Could you check a few things on this model? Use its own coordinates, in mm. Face numbers are marked on the shaded views. A direction names the side the tool comes from. Round coordinates to 2 decimals unless told otherwise and drop trailing zeros. Write each loop counter-clockwise with the first axis right and the second up, starting at its lowest first coordinate (ties: lowest second). Pieces come first, ordered by that corner, then holes. Notation, with made-up numbers: M 33,-26 L 84,-26 A19 cw 84,5 Z; hole C 25,-35 d11. An arc over 180 degrees is marked long. One line per item, written item: value. Start each with the question number.
(1) If I drill on L1, parallel to Y at x = 0, z = -8; L2, parallel to Z at x = 16.5, y = -23.5; L3, parallel to X at y = -17, z = -6, over which ranges is the centre line in solid material (lowest first)?
(2) Which directions (+Z, -Z, +X, -X, +Y, -Y) give clear straight access to the entire face, cutting with the end or side of a thin tool? Please do the marked faces 5, 6, 7, 8 and 9.
(3) I'm going to push flat-ended pins straight in: pin 1 Ø13 at (x, y) = (30.31, 17.5) entering from +Z; pin 2 Ø1.5 at (x, z) = (-36.5, 2.5) entering from +Y; pin 3 Ø1 at (y, z) = (-13.5, -5.5) entering from +X; pin 4 Ø12 at (x, z) = (26, 17.5) entering from -Y. Where does each tip first touch, or does it pass through?
(4) I want a section at A-A on z = -4. Please give me the cut outline in (x, y).
(5) I want a section at D-D on x = -11. Please give me the cut outline in (y, z), and give its area (3 significant figures).
(6) I want a section at C-C on y = 6. Please give me the cut outline in (x, z), and give its area (3 significant figures).
(7) I want a section at B-B on y = 35. Please give me the cut outline in (x, z), and give its area (3 significant figures).
(8) Thinking about a two-plate mould opening in Y: for the marked faces 1, 2, 3 and 4, which applies, released by +Y, released by -Y, zero draft, split by the parting line, or undercut?
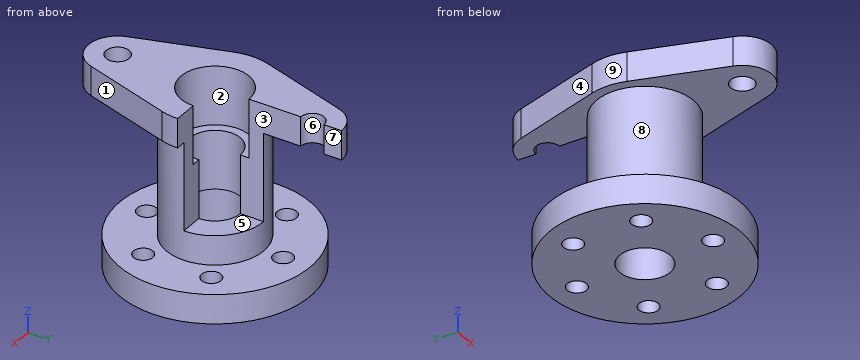
```python
from build123d import *

# Parameters (mm, degrees)
ROUND_FLANGE_SKETCH_98_R        = 49
ROUND_FLANGE_98X15_DEPTH        = 15
BOLT_HOLES_SKETCH_6X_10_PCD70_R = 5
BOLT_HOLES_6X_10_DEPTH          = 15
SLEEVE_SKETCH_50_R              = 25
SLEEVE_50X60_DEPTH              = 60
MOUNTING_FLANGE_DEPTH           = 15
SLEEVE_START                    = -60
SLEEVE_SECTION_CUT_DEPTH        = 60
SLOT_SKETCH_35X12_R             = 17.5
SLOT_SKETCH_35X12_R_2           = 6
SLOT_CUT_35X12_DEPTH            = 60
INNER_START                     = 30
INNER_BOSS_DEPTH                = 30
INNER_BORE_SKETCH_R             = 13
INNER_BORE_CUT_DEPTH            = 30


with BuildPart() as part:
    # Round Flange Sketch Ø98 → Round Flange Ø98x15 (new body)
    with BuildSketch(Plane.XY):
        Circle(ROUND_FLANGE_SKETCH_98_R)
    extrude(amount=-ROUND_FLANGE_98X15_DEPTH)

    # Bolt Holes Sketch 6xØ10 PCD70 → Bolt Holes 6xØ10 (cut)
    with BuildSketch(Plane.XY):
        with Locations((0, 35)):
            Circle(BOLT_HOLES_SKETCH_6X_10_PCD70_R)
        with Locations((30.310889132, 17.5)):
            Circle(BOLT_HOLES_SKETCH_6X_10_PCD70_R)
        with Locations((30.310889132, -17.5)):
            Circle(BOLT_HOLES_SKETCH_6X_10_PCD70_R)
        with Locations((0, -35)):
            Circle(BOLT_HOLES_SKETCH_6X_10_PCD70_R)
        with Locations((-30.310889132, -17.5)):
            Circle(BOLT_HOLES_SKETCH_6X_10_PCD70_R)
        with Locations((-30.310889132, 17.5)):
            Circle(BOLT_HOLES_SKETCH_6X_10_PCD70_R)
    extrude(amount=-BOLT_HOLES_6X_10_DEPTH, mode=Mode.SUBTRACT)

    # Sleeve Sketch Ø50 → Sleeve Ø50x60 (add)
    with BuildSketch(Plane.XY):
        Circle(SLEEVE_SKETCH_50_R)
    extrude(amount=SLEEVE_50X60_DEPTH)

    # Mounting Flange Sketch → Mounting Flange (add)
    with BuildSketch(Plane.XY.offset(60)):
        with BuildLine():
            Line((-28.618176043, -9), (-14.309088021, -54.5))
            ThreePointArc((-14.309088021, -54.5), (0, -65), (14.309088021, -54.5))
            Line((14.309088021, -54.5), (28.618176043, -9))
            ThreePointArc((28.618176043, -9), (30, 0), (28.618176043, 9))
            Line((28.618176043, 9), (14.309088021, 54.5))
            ThreePointArc((14.309088021, 54.5), (0, 65), (-14.309088021, 54.5))
            Line((-14.309088021, 54.5), (-28.618176043, 9))
            ThreePointArc((-28.618176043, 9), (-30, 0), (-28.618176043, -9))
        make_face()
    extrude(amount=MOUNTING_FLANGE_DEPTH)

    # Sleeve Section Cut Sketch → Sleeve Section Cut (cut)
    with BuildSketch(Plane.XY.offset(75).offset(SLEEVE_START)):
        with BuildLine():
            Line((0, 65), (0, 0))
            Line((0, 0), (30, 0))
            ThreePointArc((30, 0), (29.652531774, 4.552730978), (28.618176043, 9))
            Line((28.618176043, 9), (14.309088021, 54.5))
            ThreePointArc((14.309088021, 54.5), (8.874119675, 62.093386622), (0, 65))
        make_face()
    extrude(amount=SLEEVE_SECTION_CUT_DEPTH, mode=Mode.SUBTRACT)

    # Slot Sketch 35x12 → Slot Cut 35x12 (cut)
    with BuildSketch(Plane.XY.offset(75)):
        Circle(SLOT_SKETCH_35X12_R)
        with Locations((0, 50)):
            Circle(SLOT_SKETCH_35X12_R_2)
        with Locations((0, -50)):
            Circle(SLOT_SKETCH_35X12_R_2)
    extrude(amount=-SLOT_CUT_35X12_DEPTH, mode=Mode.SUBTRACT)

    # Inner Boss Sketch → Inner Boss (add)
    with BuildSketch(Plane.XY.offset(15).offset(INNER_START)):
        with BuildLine():
            Line((0, 13), (0, 17.5))
            ThreePointArc((0, 17.5), (-12.374368671, -12.374368671), (17.5, 0))
            Line((17.5, 0), (13, 0))
            ThreePointArc((13, 0), (-9.192388155, -9.192388155), (0, 13))
        make_face()
    extrude(amount=-INNER_BOSS_DEPTH)

    # Inner Bore Sketch → Inner Bore Cut (cut)
    with BuildSketch(Plane.XY.offset(15)):
        Circle(INNER_BORE_SKETCH_R)
    extrude(amount=-INNER_BORE_CUT_DEPTH, mode=Mode.SUBTRACT)


solid = part.part
```
Found:
1. L1: y = -49 to -40, -30 to -13, 13 to 30, 40 to 49
1. L2: z = -15 to 0, 60 to 75
1. L3: x = -45.96 to -35.29, -25.34 to 25.34, 35.29 to 45.96
2. face 5: +Z, +X, +Y
2. face 6: +Z, +X
2. face 7: +Z, -Z, +X, +Y
2. face 8: none
2. face 9: +Z, -X
3. pin 1: stops at z = 0
3. pin 2: passes through
3. pin 3: stops at x = 47.24
3. pin 4: stops at y = -15
4. outline: C 0,0 d98; hole C -30.31,-17.5 d10; hole C -30.31,17.5 d10; hole C 0,0 d26; hole C 0,-35 d10; hole C 0,35 d10; hole C 30.31,-17.5 d10; hole C 30.31,17.5 d10
5. outline: M -60.2,60 L -22.45,60 L -22.45,0 L -47.75,0 L -47.75,-15 L -6.93,-15 L -6.93,45 L -13.61,45 L -13.61,75 L -60.2,75 Z; M 6.93,-15 L 47.75,-15 L 47.75,0 L 22.45,0 L 22.45,60 L 60.2,60 L 60.2,75 L 13.61,75 L 13.61,45 L 6.93,45 Z
5. area: 4,280 mm²
6. outline: M -48.63,-15 L -11.53,-15 L -11.53,45 L -16.44,45 L -16.44,75 L -29.39,75 L -29.39,60 L -24.27,60 L -24.27,0 L -48.63,0 Z; M 11.53,-15 L 48.63,-15 L 48.63,0 L 24.27,0 L 24.27,15 L 11.53,15 Z
6. area: 2,190 mm²
7. outline: M -34.29,-15 L -5,-15 L -5,0 L -34.29,0 Z; M -20.44,60 L 0,60 L 0,75 L -20.44,75 Z; M 5,-15 L 34.29,-15 L 34.29,0 L 5,0 Z
7. area: 1,190 mm²
8. face 1: released by -Y
8. face 2: undercut
8. face 3: zero draft
8. face 4: released by +Y
